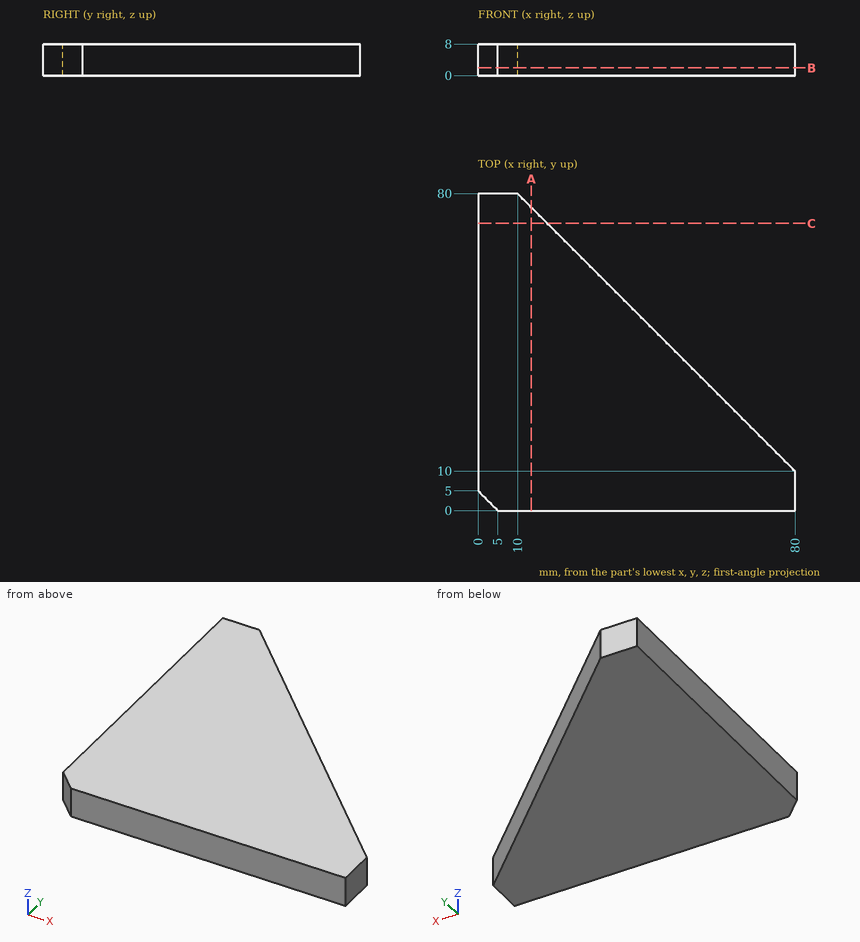
Drawing for the job (mm, zero at the part's lowest x, y, z). Coordinates: 2 decimals unless noted, no trailing zeros. Order: outer loops, then holes, each group sorted by start corner. A loop starts at its lowest first (then second) coordinate and runs counter-clockwise, first axis right, second up. Notation, with made-up numbers: (-29.5, 39.5) - (25.5, 39.5) arc R24 ccw to (25.5, 62.5) - close; hole circle Ø7 at (68.5, -36.75). An arc over 180 degrees is marked (long way). Use a Markdown table: item, result. Add a question column.
(1) Saw through at C-C (y = 72.5). Give the cut face in (x, z), then the cut area to 3 significant figures.
(2) Saw through at A-A (x = 13.5). Give the cut face in (y, z).
(3) Saw through at B-B (z = 2). Give the cut face in (x, y).
(4) Flat gauge pins, fed straight in: pin 1 (1 mm diameter, centred on y = 17.5, z = 2, fed in from +X); pin 2 (2 mm diameter, centred on y = 19.5, z = 5.5, fed in from +X); pin 3 (1 mm diameter, centred on y = 40, z = 5, fed in from +X). Where does each tip first touch, or does it go through?
(5) Drill centre lines: line 1 along X through (y, z) = (27.5, 1.5); line 2 along Y through (x, z) = (45, 1.5); line 3 along X through (y, z) = (49.5, 7.25). Where is each one in solid material? Low to high. Write a range as [from, to].
Solved:
| question | item | result |
|---|---|---|
| 1 | outline | (0, 0) - (17.5, 0) - (17.5, 8) - (0, 8) - close |
| 1 | area | 140 mm² |
| 2 | outline | (0, 0) - (76.5, 0) - (76.5, 8) - (0, 8) - close |
| 3 | outline | (0, 5) - (5, 0) - (80, 0) - (80, 10) - (10, 80) - (0, 80) - close |
| 4 | pin 1 | stops at x = 73 |
| 4 | pin 2 | stops at x = 71.5 |
| 4 | pin 3 | stops at x = 50.5 |
| 5 | line 1 | x = [0, 62.5] |
| 5 | line 2 | y = [0, 45] |
| 5 | line 3 | x = [0, 40.5] |
